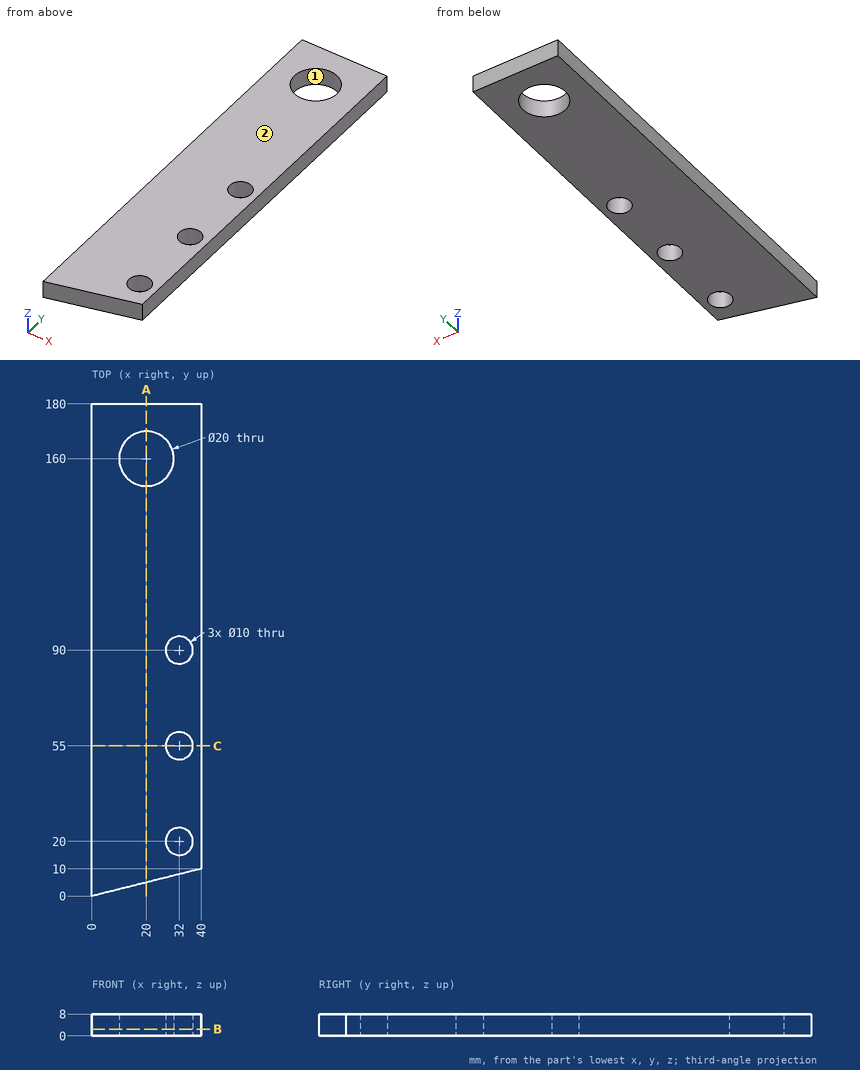
For this review, use the dimensioned drawing (mm, ordinates from the lowest corner) and the shaded views. Round coordinates to 2 decimals unless told otherwise and drop trailing zeros. Write each loop counter-clockwise with the first axis right and the second up, starting at its lowest first coordinate (ties: lowest second). Pieces come first, ordered by that corner, then holes. Notation, with made-up numbers: (-24, -16) -> (21, -16) arc R13 ccw to (21, 2) -> close; hole circle Ø10 at (75.25, 17). An arc over 180 degrees is marked (long way). Use CSV: the item, a comma, the result in double quotes.
Q1. Consider section C-C (y = 55). Give the boundary of the cut face in (x, z).
Checks:
outline,"(0, 0) -> (27, 0) -> (27, 8) -> (0, 8) -> close; (37, 0) -> (40, 0) -> (40, 8) -> (37, 8) -> close"
Q2. Mouldability with a two-part tool opening along Y and no side actions: class the marked faces 1 and 2 as released by +Y, released by -Y, zero draft, split by the parting line, or undercut.
Checks:
face 1,"undercut"
face 2,"zero draft"
Q3. For pin 1 Ø13 at (x, y) = (32, 90) entering from -Z; pin 2 Ø4 at (x, z) = (18, 4) entering from -Y, all flat-tipped, find the tip position at first contact; note any pin that passes through.
Checks:
pin 1,"z = 0"
pin 2,"y = 4"
Q4. Consider section B-B (z = 2.5). Give the boundary of the cut face in (x, y).
Checks:
outline,"(0, 0) -> (40, 10) -> (40, 180) -> (0, 180) -> close; hole circle Ø20 at (20, 160); hole circle Ø10 at (32, 20); hole circle Ø10 at (32, 55); hole circle Ø10 at (32, 90)"
Q5. To check wall thickness, follow probe 1 along Y at (x, z) = (32, 2); probe 2 along Y at (x, z) = (29, 1.5); probe 3 along Y at (x, z) = (24, 5.5). State the ranges of each line that lie inside material, in increasing order. Write a range as [from, to].
Checks:
probe 1,"[8, 15], [25, 50], [60, 85], [95, 180]"
probe 2,"[7.25, 16], [24, 51], [59, 86], [94, 155.64], [164.36, 180]"
probe 3,"[6, 150.83], [169.17, 180]"
Q6. Consider section A-A (x = 20). Give the boundary of the cut face in (y, z), then the cut area to 3 significant figures.
Checks:
outline,"(5, 0) -> (150, 0) -> (150, 8) -> (5, 8) -> close; (170, 0) -> (180, 0) -> (180, 8) -> (170, 8) -> close"
area,"1,240 mm²"
